Design review of the part built by this model. Coordinates are the model's own, in mm. Face numbers are marked on the shaded views. A direction names the side the tool comes from. Coordinates: 2 decimals unless noted, no trailing zeros. Write each loop counter-clockwise with the first axis right and the second up, starting at its lowest first coordinate (ties: lowest second). Pieces come first, ordered by that corner, then holes. Notation, with made-up numbers: (85, 25) - (131, 25) arc R26 ccw to (131, 47) - close; hole circle Ø11 at (-16, 25). An arc over 180 degrees is marked (long way). Answer as CSV lines item,"result". Start each with the question number.
Q1. We need section D-D (z = -37.5). Write out the cut boundary in (x, y), plus the area to 3 significant figures.
Q2. We need section A-A (z = -9). Write out the cut boundary in (x, y), plus the area to 3 significant figures.
Q3. Clearance check with flat-ended pins moving along their axes: pin 1 (3 mm diameter, centred on x = -2.5, z = -5, fed in from +Y); pin 2 (5 mm diameter, centred on y = 14.5, z = -36.5, fed in from +X); pin 3 (8 mm diameter, centred on y = 3.5, z = -3, fed in from +X). State where each tip first meets the part, or that it passes through.
Q4. We need section B-B (x = 0). Write out the cut boundary in (y, z), plus the area to 3 significant figures.
Q5. Machinability: for the marked faces 5, 6, 7 and 8, which of the approach directions +Z, -Z, +X, -X, +Y, -Y give a long, thin tool a straight path to every point of the face, cutting with its end or side? Answer none if there is none.
Q6. For line 1 along Z through (x, y) = (18.5, 13); line 2 along Z through (x, y) = (-15.5, 21.5); line 3 along Z through (x, y) = (14, 13.5), list the stretches that pass through material, from the lowest coordinate up. Write a range as [from, to].
Q7. We need section C-C (z = -53). Write out the cut boundary in (x, y), plus the area to 3 significant figures.
Q8. Mouldability with a two-part tool opening along Z and no side actions: class the marked faces 1, 2, 3 and 4 as pulls with the +Z half, pulls with the -Z half, needs draft (parallel to the pull), parting line crosses it, or undercut.
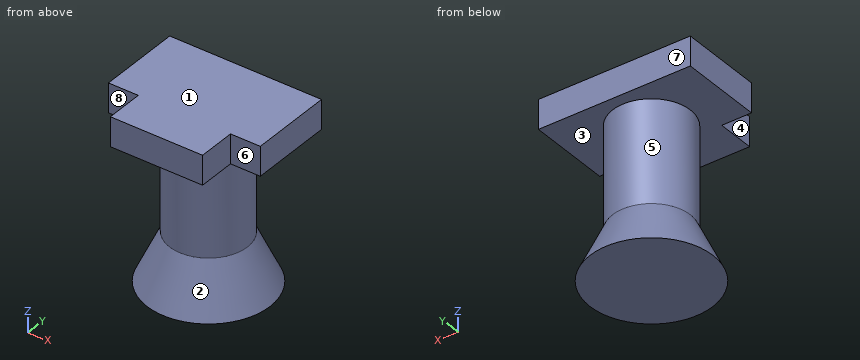
from build123d import *

# Parameters (mm, degrees)
BOSS_EXTRUDE1_DEPTH = 10
SKETCH2_R           = 13.300670815
BOSS_EXTRUDE2_DEPTH = 35


with BuildPart() as part:
    # Sketch1 → Boss-Extrude1 (new body)
    with BuildSketch(Plane.XY):
        Polygon((15.791965236, 0), (-15.791965236, 0), (-15.791965236, 12.932711507), (-25.996035407, 12.932711507), (-25.996035407, 41.33), (25.996035407, 41.33), (25.996035407, 12.932711507), (15.791965236, 12.932711507), align=None)
    extrude(amount=-BOSS_EXTRUDE1_DEPTH)

    # Sketch2 → Boss-Extrude2 (add)
    with BuildSketch(Plane(origin=(0, 0, -10), x_dir=(-1, 0, 0), z_dir=(0, 0, -1))):
        with Locations(Location((0, 24.130997224, 0), (0, 0, 180))):
            Circle(SKETCH2_R)
    extrude(amount=BOSS_EXTRUDE2_DEPTH)

    # Sketch5 → Revolve4 (revolve)
    with BuildSketch(Plane(origin=(0, 0, 0), x_dir=(0, 0, -1), z_dir=(1, 0, 0)), mode=Mode.PRIVATE) as revolve4_sk:
        Polygon((45, 37.431668039), (61.711724745, 45.151819741), (61.711724745, 24.130997224), (45, 24.130997224), align=None)
    revolve(revolve4_sk.sketch.rotate(Axis((0, 24.130997224, -45), (0, 0, -1)), 90), axis=Axis((0, 24.130997224, -45), (0, 0, -1)))


solid = part.part
Results list:
1,outline,"circle Ø26.6 at (0, 24.13)"
1,area,"556 mm2"
2,outline,"(-26, 12.93) - (-15.79, 12.93) - (-15.79, 0) - (15.79, 0) - (15.79, 12.93) - (26, 12.93) - (26, 41.33) - (-26, 41.33) - close"
2,area,"1,880 mm2"
3,pin 1,"stops at y = 41.33"
3,pin 2,"stops at x = 11.23"
3,pin 3,"stops at x = 15.79"
4,outline,"(0, -10) - (10.83, -10) - (10.83, -45) - (3.11, -61.71) - (45.15, -61.71) - (37.43, -45) - (37.43, -10) - (41.33, -10) - (41.33, 0) - (0, 0) - close"
4,area,"1,920 mm2"
5,face 5,"none"
5,face 6,"+Z, +X, -Y"
5,face 7,"+Z, +X, -X, +Y"
5,face 8,"+Z, -X, -Y"
6,line 1,"z = [-10, 0]"
6,line 2,"z = [-61.71, -50.24], [-10, 0]"
6,line 3,"z = [-61.71, -54.26], [-10, 0]"
7,outline,"circle Ø33.99 at (0, 24.13)"
7,area,"908 mm2"
8,face 1,"pulls with the +Z half"
8,face 2,"undercut"
8,face 3,"undercut"
8,face 4,"needs draft"
